Verification items for the finished model (mm, model axes). Face numbers are marked on the shaded views. Round coordinates to 2 decimals unless told otherwise and drop trailing zeros. Order: outer loops, then holes, each group sorted by start corner. A loop starts at its lowest first (then second) coordinate and runs counter-clockwise, first axis right, second up.
```python
from build123d import *

# Parameters (mm, degrees)
EXTRUDE_1_DEPTH = 850


with BuildPart() as part:
    # 草图1 → 凸台-拉伸1 (new body)
    with BuildSketch(Plane.XY.offset(425)):
        with BuildLine():
            Line((2520.186202106, 858.855453105), (3516.380900198, 771.699710358))
            ThreePointArc((3516.380900198, 771.699710358), (3573.650354384, 703.448632585), (3505.399276611, 646.179178398))
            Line((3505.399276611, 646.179178398), (2509.20457852, 733.334921146))
            ThreePointArc((2509.20457852, 733.334921146), (2451.935124333, 801.585998919), (2520.186202106, 858.855453105))
        make_face()
        with BuildLine():
            Line((2519.924734878, 855.866869011), (3516.119432969, 768.711126263))
            ThreePointArc((3516.119432969, 768.711126263), (3570.66177029, 703.710099813), (3505.66074384, 649.167762492))
            Line((3505.66074384, 649.167762492), (2509.466045748, 736.32350524))
            ThreePointArc((2509.466045748, 736.32350524), (2454.923708427, 801.32453169), (2519.924734878, 855.866869011))
        make_face(mode=Mode.SUBTRACT)
    extrude(amount=-EXTRUDE_1_DEPTH)


solid = part.part
```
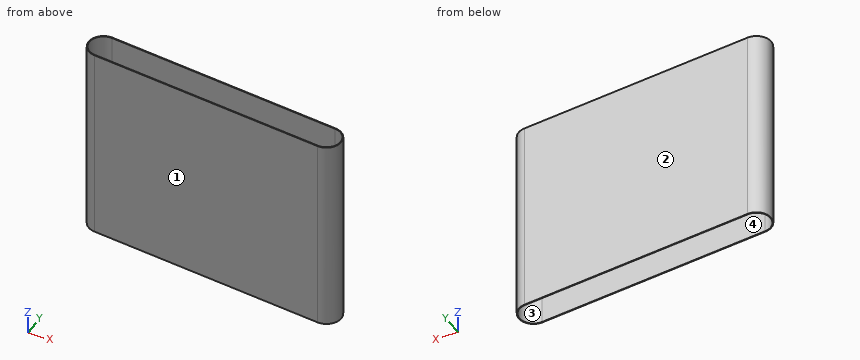
1) Scan lines: probe 1 along Y at (x, z) = (3290.5, 391); probe 2 along Y at (x, z) = (3338.5, -86.5); probe 3 along X at (y, z) = (751.5, -31). Record each from-to range of solid material in increasing order.
2) Go/stop test with flat-tipped pins: pin 1 Ø8 at (x, z) = (3200.5, 185.5) entering from +Y; pin 2 Ø8 at (y, z) = (756.5, 273.5) entering from +X; pin 3 Ø8 at (x, z) = (3305, -317.5) entering from -Y. Record where each tip stops, or that it passes through.
3) Draft check along X on the marked faces 1, 2, 3 and 4. Enter one of: released by +X, released by -X, zero draft, split by the parting line, or undercut.
4) Sectioned sample at C-C on x = 2612. Record the cut outline in (y, z).
5) Sectioned sample at B-B on y = 805.5. Record the cut outline in (x, z), then the cut area to 3 significant figures.
6) Sectioned sample at A-A on z = 236. Record the cut outline in (x, y), then the cut area to 3 significant figures.
Returned:
1. probe 1: y = 664.98 to 667.99, 788.45 to 791.46
1. probe 2: y = 660.78 to 663.79, 784.25 to 787.26
1. probe 3: x = 2470.2 to 2474.55, 3553.18 to 3557.34
2. pin 1: stops at y = 799.69
2. pin 2: stops at x = 3556.4
2. pin 3: stops at y = 663.36
3. face 1: released by -X
3. face 2: released by +X
3. face 3: undercut
3. face 4: undercut
4. outline: (724.34, -425) - (727.35, -425) - (727.35, 425) - (724.34, 425) - close; (847.81, -425) - (850.82, -425) - (850.82, 425) - (847.81, 425) - close
5. outline: (2452.4, -425) - (2455.44, -425) - (2455.44, 425) - (2452.4, 425) - close; (3095.62, -425) - (3130.04, -425) - (3130.04, 425) - (3095.62, 425) - close
5. area: 31,800 mm2
6. outline: (2509.2, 733.33) - (3505.4, 646.18) arc R63 ccw to (3516.38, 771.7) - (2520.19, 858.86) arc R63 ccw to start; hole (2509.47, 736.32) - (3505.66, 649.17) arc R60 ccw to (3516.12, 768.71) - (2519.92, 855.87) arc R60 ccw to start
6. area: 7,160 mm2
